Input: part model. Units: mm. Frame: model coordinates. A direction names the side the tool comes from. Round coordinates to 2 decimals unless told otherwise and drop trailing zeros. Loops run counter-clockwise (first coordinate to the right, second up) from the corner with the lowest first, then second, coordinate; pieces in that order, holes last. Notation, with made-up numbers: (-37.5, 27) - (-28.5, 27) arc R14 cw to (-28.5, 32) - close; hole circle Ø8 at (54.5, 1). An arc over 180 degrees is marked (long way). Write each question's results on one line, items separated by ' | '.
from build123d import *

# Parameters (mm, degrees)
MAIN_BARREL_28_DEPTH      = 17.5
MAIN_BARREL_28_DEPTH_BACK = 17.5
MAIN_BARREL_SKETCH_R      = 14
MAIN_BORE_SKETCH_R        = 9
MAIN_BORE_18_DEPTH        = 41.211938526
UPPER_BOSS_SKETCH_R       = 7.5
UPPER_BOSS_15_DEPTH       = 9.5
UPPER_BORE_SKETCH_R       = 4.5
UPPER_BORE_9_DEPTH        = 45.505617623
CONNECTING_WEB_DEPTH      = 2.5


with BuildPart() as part:
    # Main Barrel Sketch → Main Barrel _28 (new, two sides: drawn at the far end of the back side and taken through both)
    with BuildSketch(Plane.XY.offset(-MAIN_BARREL_28_DEPTH_BACK)):
        Circle(MAIN_BARREL_SKETCH_R)
    extrude(amount=MAIN_BARREL_28_DEPTH + MAIN_BARREL_28_DEPTH_BACK)

    # Main Bore Sketch → Main Bore _18 (cut, through all)
    with BuildSketch(Plane.XY.offset(17.5)):
        Circle(MAIN_BORE_SKETCH_R)
    extrude(amount=-MAIN_BORE_18_DEPTH, mode=Mode.SUBTRACT)



with BuildPart() as body_2:
    # Upper Boss Sketch → Upper Boss _15 (new, symmetric)
    with BuildSketch(Plane(origin=(0, 0, 0), x_dir=(0, 0, -1), z_dir=(1, 0, 0))):
        with Locations((0, 26)):
            Circle(UPPER_BOSS_SKETCH_R)
    extrude(amount=UPPER_BOSS_15_DEPTH, both=True)

    # Upper Bore Sketch → Upper Bore _9 (cut, through all)
    with BuildSketch(Plane(origin=(9.5, 0, 0), x_dir=(0, 0, -1), z_dir=(1, 0, 0))):
        with Locations((0, 26)):
            Circle(UPPER_BORE_SKETCH_R)
    extrude(amount=-UPPER_BORE_9_DEPTH, mode=Mode.SUBTRACT)


with BuildPart() as part_1:
    add(part.part)

    add(body_2.part)  # Connecting Web merges body 2
    # Web Sketch → Connecting Web (add, symmetric)
    with BuildSketch(Plane(origin=(0, 0, 0), x_dir=(0, 0, -1), z_dir=(1, 0, 0))):
        with BuildLine():
            Line((-6.153967777, 30.287036342), (-17.5, 14))
            Line((-17.5, 14), (-17.5, 13))
            Line((-17.5, 13), (17.5, 13))
            Line((17.5, 13), (17.5, 14))
            Line((17.5, 14), (6.153967777, 30.287036342))
            ThreePointArc((6.153967777, 30.287036342), (7.155583775, 28.246691086), (7.5, 26))
            ThreePointArc((7.5, 26), (-2.246691086, 18.844416225), (-6.153967777, 30.287036342))
        make_face()
    extrude(amount=CONNECTING_WEB_DEPTH, both=True)


solid = part_1.part
1. Contact query for flat-ended pins moving along their axis: pin 1 (4 mm diameter, centred on x = -5, z = 10, fed in from -Y); pin 2 (16.5 mm diameter, centred on y = 29, z = -2.5, fed in from +X); pin 3 (5 mm diameter, centred on x = 7.5, y = 20, fed in from -Z). Output: stop coordinate, or through.
Answer:
pin 1: y = -13.67 | pin 2: x = 9.5 | pin 3: z = -6.63
2. Section query A-A, the plane z = 0. Output: boundary loops of the cut face in (x, y).
Answer:
outline: (-9.5, 18.5) - (-2.5, 18.5) - (-2.5, 13.77) arc R14 ccw (long way) to (2.5, 13.77) - (2.5, 18.5) - (9.5, 18.5) - (9.5, 21.5) - (-9.5, 21.5) - close; (-9.5, 30.5) - (9.5, 30.5) - (9.5, 33.5) - (-9.5, 33.5) - close; hole circle Ø18 at (0, 0)
3. Section query C-C, the plane x = 5. Output: boundary loops of the cut face in (y, z), plus the area to 3 significant figures.
Answer:
outline: (-13.08, -17.5) - (-7.48, -17.5) - (-7.48, 17.5) - (-13.08, 17.5) - close; (7.48, -17.5) - (13.08, -17.5) - (13.08, 17.5) - (7.48, 17.5) - close; circle Ø15 at (26, 0); hole circle Ø9 at (26, 0) | area: 505 mm^2
4. Line query: line 1 (Y direction, x = 8.25, z = 6.5); line 2 (Y direction, x = 0, z = -4); line 3 (X direction, y = 15.5, z = -15.5). Output: solid intervals per line, ascending. Write a range as [from, to].
Answer:
line 1: [-11.31, -3.6], [3.6, 11.31], [22.26, 29.74] | line 2: [-14, -9], [9, 23.94], [28.06, 32.34] | line 3: [-2.5, 2.5]
5. Set-up query: faces 4 (the flat face through (-9.5, 26, -5)), 5 (the flat face through (2.5, 18, 0)), 6 (the cylindrical face through (-0.58, -13.988, -0.245)), 7 (the cylindrical face through (0.133, 33.436, 0.976)). Return all of +Z, -Z, +X, -X, +Y, -Y with unobstructed straight access to the full face (end or side cutting, diameter ignored); none if empty.
Answer:
face 4: +Z, -Z, -X, +Y | face 5: +X | face 6: +Z, -Z | face 7: none
6. Section query B-B, the plane y = 0. Output: boundary loops of the cut face in (x, z).
Answer:
outline: (-14, -17.5) - (-9, -17.5) - (-9, 17.5) - (-14, 17.5) - close; (9, -17.5) - (14, -17.5) - (14, 17.5) - (9, 17.5) - close
7. Section query D-D, the plane x = 0.75. Output: boundary loops of the cut face in (y, z).
Answer:
outline: (-13.98, -17.5) - (-8.97, -17.5) - (-8.97, 17.5) - (-13.98, 17.5) - close; (8.97, -17.5) - (14, -17.5) - (30.29, -6.15) arc R7.5 ccw to (30.29, 6.15) - (14, 17.5) - (8.97, 17.5) - close; hole circle Ø9 at (26, 0)
8. Mould query, pull axis Y, two halves, no side actions, for faces 1 (the flat face through (9.5, 26, -5)), 2 (the flat face through (-2.5, 18, 0)), 3 (the flat face through (0.035, 22.258, 11.748)). Classes: pulls with the +Y half, pulls with the -Y half, needs draft (parallel to the pull), parting line crosses it, or undercut.
Answer:
face 1: needs draft | face 2: undercut | face 3: pulls with the +Y half
